```python
from build123d import *

# Parameters (mm, degrees)
LEG_PLATE_10MM_DEPTH = 5


with BuildPart() as part:
    # Leg Profile Sketch → Leg Plate 10mm (new, symmetric)
    with BuildSketch(Plane.XY):
        Polygon((0, 0), (113.589838486, 0), (108.230854638, 20), (88.230854638, 20), (88.230854638, 30), (105.551362713, 30), (86.794919243, 100), (66.794919243, 100), (66.794919243, 110), (46.794919243, 110), (46.794919243, 100), (26.794919243, 100), (18.75644347, 70), (36.076951546, 70), (36.076951546, 60), (16.076951546, 60), align=None)
    extrude(amount=LEG_PLATE_10MM_DEPTH, both=True)


solid = part.part
```
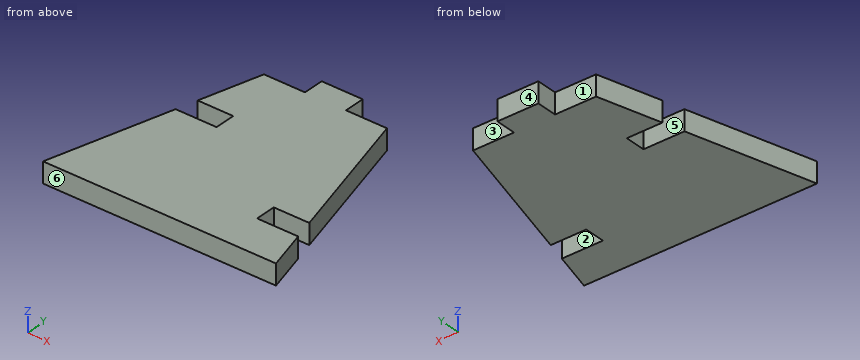
For this review, take the finished solid that the model builds, in its own axes (mm). Face numbers are marked on the shaded views. A direction names the side the tool comes from. Round coordinates to 2 decimals unless told otherwise and drop trailing zeros. Loops run counter-clockwise (first coordinate to the right, second up) from the corner with the lowest first, then second, coordinate; pieces in that order, holes last.
Q1. Mouldability with a two-part tool opening along Y and no side actions: class the marked faces 4, 5 and 6 as +Y half, -Y half, draft (parallel to the pull), parting line (faces both ways), or undercut.
Result sheet:
face 4: +Y half
face 5: undercut
face 6: -Y half
Q2. Add section B-B on z = 0.75. Write out the cut boundary in (x, y), plus the area to 3 significant figures.
Result sheet:
outline: (0, 0) - (113.59, 0) - (108.23, 20) - (88.23, 20) - (88.23, 30) - (105.55, 30) - (86.79, 100) - (66.79, 100) - (66.79, 110) - (46.79, 110) - (46.79, 100) - (26.79, 100) - (18.76, 70) - (36.08, 70) - (36.08, 60) - (16.08, 60) - close
area: 8,510 mm2
Q3. Add section C-C on x = 80.5. Write out the cut boundary in (y, z).
Result sheet:
outline: (0, -5) - (100, -5) - (100, 5) - (0, 5) - close
Q4. Machinability: for the marked faces 1, 2 and 3, which of the approach directions +Z, -Z, +X, -X, +Y, -Y give a long, thin tool a straight path to every point of the face, cutting with its end or side? Answer none if there is none.
Result sheet:
face 1: +Z, -Z, -X, +Y
face 2: +Z, -Z, +X
face 3: +Z, -Z, +X, +Y
Q5. Insertion check: pin 1 Ø3 at (y, z) = (107, -2.5) entering from -X; pin 2 Ø5 at (y, z) = (47, 1.5) entering from +X; pin 3 Ø5 at (x, z) = (34.5, 1) entering from +Y. Each pin has a flat end and moves straight along its axis. Give the tip position at first contact, or say it passes through.
Result sheet:
pin 1: stops at x = 46.79
pin 2: stops at x = 101.67
pin 3: stops at y = 100
Q6. Add section A-A on x = 34.5. Write out the cut boundary in (y, z).
Result sheet:
outline: (0, -5) - (60, -5) - (60, 5) - (0, 5) - close; (70, -5) - (100, -5) - (100, 5) - (70, 5) - close
Q7. Add section D-D on y = 57.5. Write out the cut boundary in (x, z).
Result sheet:
outline: (15.41, -5) - (98.18, -5) - (98.18, 5) - (15.41, 5) - close
Q8. To check wall thickness, follow line 1 along Y through (x, z) = (18, -2); line 2 along Y through (x, z) = (86, -1.5); line 3 along X through (y, z) = (29, -3.25). State the ranges of each line that lie inside material, in increasing order.
Result sheet:
line 1: y = 0 to 60
line 2: y = 0 to 100
line 3: x = 7.77 to 88.23
